Here's how the part is built. I have some questions about the finished solid (model axes, mm). Give positions to 0.01 mm unless a question says otherwise; leave off trailing zeros. Write each loop counter-clockwise with the first axis right and the second up, starting at its lowest first coordinate (ties: lowest second). Pieces come first, ordered by that corner, then holes. Notation, with made-up numbers: (-4.75, -6) -> (51.25, -6) arc R10 cw to (51.25, 0) -> close; hole circle Ø5 at (36.25, -7). An arc over 180 degrees is marked (long way). Return JSON: item names as keys, results as strings.
from build123d import *

# Parameters (mm, degrees)
SKETCH1_R           = 3.5
SKETCH1_R_2         = 4.5
SKETCH1_R_3         = 4
BOSS_EXTRUDE1_DEPTH = 5
FILLET1_R           = 2
FILLET2_R           = 5


with BuildPart() as part:
    # Sketch1 → Boss-Extrude1 (new body)
    with BuildSketch(Plane.XY):
        with BuildLine():
            Line((8.964694833, 90), (9.516445583, 79.471968525))
            ThreePointArc((9.516445583, 79.471968525), (19.681156059, 68.23864229), (32.744762205, 75.910092728))
            ThreePointArc((32.744762205, 75.910092728), (37.408516237, 78.659737666), (42.755349998, 77.809727269))
            Line((42.755349998, 77.809727269), (52.755349998, 72.309727269))
            ThreePointArc((52.755349998, 72.309727269), (56.88996042, 65.700665064), (53.437266153, 58.711129395))
            Line((53.437266153, 58.711129395), (46.88062952, 54.196060385))
            ThreePointArc((46.88062952, 54.196060385), (45.131399706, 52.224869926), (44.5, 49.666211844))
            Line((44.5, 49.666211844), (44.5, 0))
            Line((44.5, 0), (0, 0))
            Line((0, 0), (0, 90))
            Line((0, 90), (8.964694833, 90))
        make_face()
        with Locations((48.9, 65.3)):
            Circle(SKETCH1_R, mode=Mode.SUBTRACT)
        with Locations((10, 10)):
            Circle(SKETCH1_R_2, mode=Mode.SUBTRACT)
        with Locations((10, 25)):
            Circle(SKETCH1_R_3, mode=Mode.SUBTRACT)
        with Locations((34.5, 10)):
            Circle(SKETCH1_R_3, mode=Mode.SUBTRACT)
        with Locations((34.5, 25)):
            Circle(SKETCH1_R_2, mode=Mode.SUBTRACT)
        with Locations((23, 50.5)):
            Circle(SKETCH1_R, mode=Mode.SUBTRACT)
    extrude(amount=BOSS_EXTRUDE1_DEPTH)

    # Fillet1
    fillet1_edges = [part.edges().sort_by_distance(p)[0] for p in [
        (0, 90, 2.5),
        (8.964694833, 90, 2.5),
    ]]
    fillet(fillet1_edges, radius=FILLET1_R)

    # Fillet2
    fillet2_edges = [part.edges().sort_by_distance(p)[0] for p in [
        (44.5, 0, 2.5),
        (0, 0, 2.5),
    ]]
    fillet(fillet2_edges, radius=FILLET2_R)


solid = part.part
1. Suppose I cut it at B-B, the plane y = 65.3. List the corners of the cut face in (x, z) for me.
Taken from the geometry:
{"outline": "(0, 0) -> (45.4, 0) -> (45.4, 5) -> (0, 5) -> close; (52.4, 0) -> (56.9, 0) -> (56.9, 5) -> (52.4, 5) -> close"}
2. If I drill on line 1 (Y direction, x = 34.5, z = 1.3); line 2 (X direction, y = 10.5, z = 3.6); line 3 (Y direction, x = 37.5, z = 4.05), over which ranges is the centre line in solid material (lowest first)? Write a range as [from, to].
Taken from the geometry:
{"line 1": "y = [0, 6], [14, 20.5], [29.5, 77.48]", "line 2": "x = [0, 5.53], [14.47, 30.53], [38.47, 44.5]", "line 3": "y = [0, 7.35], [12.65, 21.65], [28.35, 78.68]"}
3. If we mould it in two halves opening along Y, with no side actions, what happens to faces 1 (the face through (23, 54, 2)), 2 (the face through (47.685, 75.098, 2.465)), 3 (the face through (1, 2, 3))? For each: released by +Y, released by -Y, zero draft, split by the parting line, or undercut.
Taken from the geometry:
{"face 1": "undercut", "face 2": "released by +Y", "face 3": "released by -Y"}
4. Suppose I cut it at A-A, the plane z = 4.15. List the corners of the cut face in (x, y) for me.
Taken from the geometry:
{"outline": "(0, 5) arc R5 ccw to (5, 0) -> (39.5, 0) arc R5 ccw to (44.5, 5) -> (44.5, 49.67) arc R5.5 cw to (46.88, 54.2) -> (53.44, 58.71) arc R8 ccw to (52.76, 72.31) -> (42.76, 77.81) arc R8 ccw to (32.74, 75.91) arc R12 cw to (9.52, 79.47) -> (9.06, 88.1) arc R2 ccw to (7.07, 90) -> (2, 90) arc R2 ccw to (0, 88) -> close; hole circle Ø9 at (10, 10); hole circle Ø8 at (10, 25); hole circle Ø7 at (23, 50.5); hole circle Ø9 at (34.5, 25); hole circle Ø8 at (34.5, 10); hole circle Ø7 at (48.9, 65.3)"}
5. For pin 1 Ø8 at (x, y) = (10, 10) entering from +Z; pin 2 Ø2.5 at (y, z) = (37.5, 1.5) entering from +X, each with a flat end and sliding along its axis, tell me the tip position at first contact or that it passes through.
Taken from the geometry:
{"pin 1": "passes through", "pin 2": "stops at x = 44.5"}
6. Suppose I cut it at C-C, the plane x = 48.9. List the corners of the cut face in (y, z) for me.
Taken from the geometry:
{"outline": "(55.59, 0) -> (61.8, 0) -> (61.8, 5) -> (55.59, 5) -> close; (68.8, 0) -> (74.43, 0) -> (74.43, 5) -> (68.8, 5) -> close"}
7. Suppose I cut it at D-D, the plane x = 34.5. List the corners of the cut face in (y, z) for me.
Taken from the geometry:
{"outline": "(0, 0) -> (6, 0) -> (6, 5) -> (0, 5) -> close; (14, 0) -> (20.5, 0) -> (20.5, 5) -> (14, 5) -> close; (29.5, 0) -> (77.48, 0) -> (77.48, 5) -> (29.5, 5) -> close"}
